Can you work these out from the model? Positions are in its coordinate system, mm. A direction names the side the tool comes from. Round coordinates to 2 decimals unless told otherwise and drop trailing zeros. Loops run counter-clockwise (first coordinate to the right, second up) from the corner with the lowest first, then second, coordinate; pieces in that order, holes last. Notation, with made-up numbers: M 21,47 L 54,47 A26 cw 54,70 Z; hole C -38,-12.5 d4. An arc over 180 degrees is marked long. Return JSON: item names as keys, results as strings.
```python
from build123d import *

# Parameters (mm, degrees)
BOSS_EXTRUDE1_DEPTH = 1000


with BuildPart() as part:
    # Sketch2 → Boss-Extrude1 (new, symmetric)
    with BuildSketch(Plane(origin=(0, 0, 0), x_dir=(1, 0, 0), z_dir=(0, 1, 0))):
        with BuildLine():
            Line((7.875, -1.525), (92.125, -1.525))
            ThreePointArc((92.125, -1.525), (97.693465902, 0.781534098), (100, 6.35))
            Line((100, 6.35), (100, 90.6))
            ThreePointArc((100, 90.6), (97.693465902, 96.168465902), (92.125, 98.475))
            Line((92.125, 98.475), (7.875, 98.475))
            ThreePointArc((7.875, 98.475), (2.306534098, 96.168465902), (0, 90.6))
            Line((0, 90.6), (0, 6.35))
            ThreePointArc((0, 6.35), (2.306534098, 0.781534098), (7.875, -1.525))
        make_face()
        with BuildLine():
            Line((12.6, 4.775), (87.4, 4.775))
            ThreePointArc((87.4, 4.775), (91.854772721, 6.620227279), (93.7, 11.075))
            Line((93.7, 11.075), (93.7, 85.875))
            ThreePointArc((93.7, 85.875), (91.854772721, 90.329772721), (87.4, 92.175))
            Line((87.4, 92.175), (12.6, 92.175))
            ThreePointArc((12.6, 92.175), (8.145227279, 90.329772721), (6.3, 85.875))
            Line((6.3, 85.875), (6.3, 11.075))
            ThreePointArc((6.3, 11.075), (8.145227279, 6.620227279), (12.6, 4.775))
        make_face(mode=Mode.SUBTRACT)
    extrude(amount=BOSS_EXTRUDE1_DEPTH, both=True)


solid = part.part
```
Q1. On a 3-axis mill with a long thin cutter (end or side, diameter ignored), from which of +Z, -Z, +X, -X, +Y, -Y can I reach the whole of each face in a straight line? I mean faces 1 (the flat face through (93.7, 14, -48)), 2 (the flat face through (94, 1000, -49)). Say none if no direction works.
Results:
{"face 1": "+Y, -Y", "face 2": "+Z, -Z, +X, -X, +Y"}
Q2. Thinking about a two-plate mould opening in Z: for faces 3 (the flat face through (100, 14, -48)), 4 (the flat face through (49, 14, 1.525)), 5 (the flat face through (51, 14, -92.175)), which applies, pulls with the +Z half, pulls with the -Z half, needs draft (parallel to the pull), parting line crosses it, or undercut?
Results:
{"face 3": "needs draft", "face 4": "pulls with the +Z half", "face 5": "undercut"}
Q3. If I drill on line 1 along Z through (x, y) = (53, -142.5) (3 decimals); line 2 along X through (y, z) = (-304, -38.5); line 3 along Z through (x, y) = (7.5, -603.5), over which ranges is the centre line in solid material (lowest first)?
Results:
{"line 1": "z = -98.475 to -92.175, -4.775 to 1.525", "line 2": "x = 0 to 6.3, 93.7 to 100", "line 3": "z = -98.47 to -89.57, -7.38 to 1.52"}
Q4. Suppose I cut it at B-B, the plane x = 28. Please give me the cut outline in (y, z) (3 decimals).
Results:
{"outline": "M -1000,-98.475 L 1000,-98.475 L 1000,-92.175 L -1000,-92.175 Z; M -1000,-4.775 L 1000,-4.775 L 1000,1.525 L -1000,1.525 Z"}
Q5. Suppose I cut it at C-C, the plane y = 357.5. Please give me the cut outline in (x, z) (3 decimals), plus the area to 3 significant figures.
Results:
{"outline": "M 0,-90.6 A7.875 ccw 7.875,-98.475 L 92.125,-98.475 A7.875 ccw 100,-90.6 L 100,-6.35 A7.875 ccw 92.125,1.525 L 7.875,1.525 A7.875 ccw 0,-6.35 Z; hole M 6.3,-85.875 A6.3 ccw 12.6,-92.175 L 87.4,-92.175 A6.3 ccw 93.7,-85.875 L 93.7,-11.075 A6.3 ccw 87.4,-4.775 L 12.6,-4.775 A6.3 ccw 6.3,-11.075 Z", "area": "2,340 mm2"}
Q6. Suppose I cut it at A-A, the plane z = -47. Please give me the cut outline in (x, y), plus the area to 3 significant figures.
Results:
{"outline": "M 0,-1000 L 6.3,-1000 L 6.3,1000 L 0,1000 Z; M 93.7,-1000 L 100,-1000 L 100,1000 L 93.7,1000 Z", "area": "25,200 mm2"}
